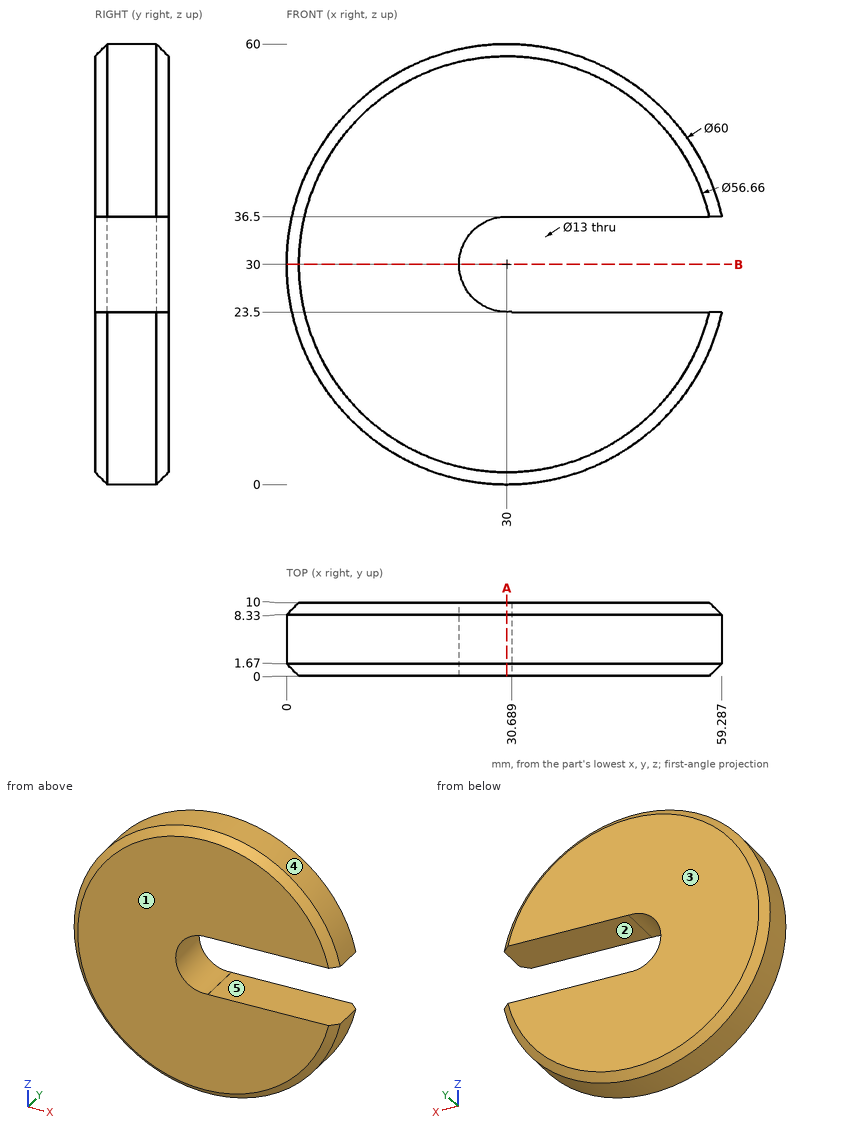
Print and shaded views of the part. All mm, measured from the part's lowest x, y and z. A direction names the side the tool comes from. Coordinates: 2 decimals unless noted, no trailing zeros. Write each loop counter-clockwise with the first axis right and the second up, starting at its lowest first coordinate (ties: lowest second). Pieces come first, ordered by that corner, then holes.
(1) Cut at A-A, the plane x = 30. List the corners of the cut face in (y, z).
(2) Flat gauge pins, fed straight in: pin 1 (1.5 mm diameter, centred on x = 19.5, y = 2, fed in from +Z); pin 2 (5 mm diameter, centred on x = 40.5, y = 5.5, fed in from -Z); pin 3 (5 mm diameter, centred on x = 49.5, y = 3, fed in from +Z); pin 4 (21 mm diameter, centred on x = 30, z = 30, fed in from -Y). Where does each tip first touch, or does it go through?
(3) Two-plate mould, pull along Z, no slides. Class the marked faces 3, 4 and 5: +Z half, -Z half, draft (parallel to the pull), parting line (faces both ways), or undercut.
(4) Drill centre lines: probe 1 along Z at (x, y) = (30, 5.5); probe 2 along X at (y, z) = (3, 30); probe 3 along Z at (x, y) = (46, 3.25). Where is each one in solid material? Low to high.
(5) 3-axis set-ups, long thin cutter, end or side, ignore diameter. For the marked faces 1 and 2: which of +Z, -Z, +X, -X, +Y, -Y reach the whole face in a straight line?
(6) Cut at B-B, the plane z = 30. List the corners of the cut face in (x, y), and give its area (3 significant figures).
Geometry says:
1. outline: (0, 1.67) - (1.67, 0) - (8.33, 0) - (10, 1.67) - (10, 23.5) - (0, 23.5) - close; (0, 36.5) - (10, 36.5) - (10, 58.33) - (8.33, 60) - (1.67, 60) - (0, 58.33) - close
2. pin 1: stops at z = 58.37
2. pin 2: stops at z = 1.09
2. pin 3: stops at z = 54.72
2. pin 4: stops at y = 0
3. face 3: draft
3. face 4: parting line
3. face 5: undercut
4. probe 1: z = 0 to 23.5, 36.5 to 60
4. probe 2: x = 0 to 23.5
4. probe 3: z = 4.62 to 23.5, 36.5 to 55.38
5. face 1: +Z, -Z, +X, -X, -Y
5. face 2: +X, +Y, -Y
6. outline: (0, 1.67) - (1.67, 0) - (23.5, 0) - (23.5, 10) - (1.67, 10) - (0, 8.33) - close
6. area: 232 mm2
